Geometry check sheet. Reference: the model listing, model coordinates, mm. A direction names the side the tool comes from. Round coordinates to 2 decimals unless told otherwise and drop trailing zeros. Order: outer loops, then holes, each group sorted by start corner. A loop starts at its lowest first (then second) coordinate and runs counter-clockwise, first axis right, second up. Notation, with made-up numbers: (63.5, 47) - (80.5, 47) arc R23 cw to (80.5, 68) - close; hole circle Ø8 at (-34.5, 79). An arc over 180 degrees is marked (long way). Return JSON: item names as keys, results as strings. Group by question number.
Q1. Material ranges on line 1 along X through (y, z) = (-109, -12); line 2 along Y through (x, z) = (-37, -4); line 3 along X through (y, z) = (110, -22), recorded low to high.
Q2. Tool access check on faces 5 (the cylindrical face through (190.764, -60.075, -37.395)), 6 (the cylindrical face through (181.35, -165.81, -9.86)), 7 (the cylindrical face through (82.598, 158.804, -7.098)). Record the directions out of +Z, -Z, +X, -X, +Y, -Y that give a thin tool (end or side, any length) a straight path to the whole face; none if there is none.
Q3. Draft check along X on faces 1 (the cylindrical face through (-174.681, 162.336, -9.86)), 2 (the flat face through (-41, 219, -20)), 3 (the cylindrical face through (-214.263, 164.291, -10.14)), 4 (the cylindrical face through (-1.432, 255.906, -9.86)). Enter one of: pulls with the +X half, pulls with the -X half, needs draft (parallel to the pull), parting line crosses it, or undercut.
Q4. Sectioned sample at B-B, the plane y = 245. Record the cut outline in (x, z).
Q5. Gauge pin test, flat ends, axial feed: pin 1 Ø10 at (x, y) = (161, 19.5) entering from -Z; pin 2 Ø10 at (x, z) = (-94, -7.5) entering from -Y; pin 3 Ø10 at (x, z) = (158.5, -30.5) entering from -Y. Record the tip position at first contact, or that the pin passes through.
```python
from build123d import *

# Parameters (mm, degrees)
SKETCH2_R          = 11
CUT_EXTRUDE1_DEPTH = 41
CIRPATTERN1_COUNT  = 8


with BuildPart() as part:
    # Sketch1 → Revolve1 (revolve)
    with BuildSketch(Plane(origin=(0, 0, 0), x_dir=(0, 0, -1), z_dir=(1, 0, 0)), mode=Mode.PRIVATE) as revolve1_sk:
        Polygon((0, 141), (0, 153), (14, 153), (14, 167), (0, 167), (0, 179), (14, 179), (14, 193), (0, 193), (0, 270), (20, 270), (20, 220), (45, 220), (45, 200), (30, 200), (30, 141), align=None)
    revolve(revolve1_sk.sketch.rotate(Axis((0, 0, 0), (0, 0, -1)), 90), axis=Axis((0, 0, 0), (0, 0, -1)))

    # Sketch2 → Cut-Extrude1 (cut)
    with BuildSketch(Plane.XY):
        with Locations((0, 245)):
            Circle(SKETCH2_R)
    cut_extrude1 = extrude(amount=-CUT_EXTRUDE1_DEPTH, mode=Mode.SUBTRACT)

    # CirPattern1: Cut-Extrude1 ×8 about axis
    cirpattern1_axis = Axis((0, 0, 0), (0, 0, 1))
    for i in range(1, CIRPATTERN1_COUNT):
        add(cut_extrude1.rotate(cirpattern1_axis, i * 360 / CIRPATTERN1_COUNT), mode=Mode.SUBTRACT)


solid = part.part
```
Reply:
{
 "1": {"line 1": "-247.02 to -159.27, -141.99 to -126.52, -107.37 to -89.44, 89.44 to 107.37, 126.52 to 141.99, 159.27 to 247.02", "line 2": "-267.45 to -189.42, -175.13 to -162.85, -148.46 to -136.06, 136.06 to 148.46, 162.85 to 175.13, 189.42 to 267.45", "line 3": "-190.53 to -88.21, 88.21 to 190.53"},
 "2": {"face 5": "-Z", "face 6": "+Z, -Z", "face 7": "+Z"},
 "3": {"face 1": "undercut", "face 2": "needs draft", "face 3": "parting line crosses it", "face 4": "undercut"},
 "4": {"outline": "(-113.47, -20) - (-11, -20) - (-11, 0) - (-113.47, 0) - close; (11, -20) - (113.47, -20) - (113.47, 0) - (11, 0) - close"},
 "5": {"pin 1": "z = -30", "pin 2": "y = -254.91", "pin 3": "y = -157.6"}
}
